Work out the finished part from the listing and answer in its coordinate system (mm). Round coordinates to 2 decimals unless told otherwise and drop trailing zeros. Order: outer loops, then holes, each group sorted by start corner. A loop starts at its lowest first (then second) coordinate and runs counter-clockwise, first axis right, second up. Notation, with made-up numbers: (84, 81.5) -> (88, 81.5) arc R36 cw to (88, 118.5) -> close; hole circle Ø6 at (40.5, 8). An arc over 180 degrees is marked (long way). Use one line per item in the form item = value.
```python
from build123d import *

# Parameters (mm, degrees)
SKETCH11_R          = 2.5
MEMBER_1_DEPTH      = 805
CUT_EXTRUDE_1_DEPTH = 404.058618566
HOLE_WIZARD_M6_1_D  = 5


with BuildPart() as part:
    # Sketch11 → Member 1 (new body)
    with BuildSketch(Plane(origin=(-402.5, 0, 0), x_dir=(0, 0, -1), z_dir=(1, 0, 0))):
        with BuildLine():
            Line((-6, -15), (-3.25, -15))
            Line((-3.25, -15), (-3.25, -12.7))
            Line((-3.25, -12.7), (-5, -12.7))
            Line((-5, -12.7), (-5, -7))
            ThreePointArc((-5, -7), (0, -4.31662479), (5, -7))
            Line((5, -7), (5, -12.7))
            Line((5, -12.7), (3.25, -12.7))
            Line((3.25, -12.7), (3.25, -15))
            Line((3.25, -15), (6, -15))
            ThreePointArc((6, -15), (7.060660172, -14.560660172), (7.5, -13.5))
            Line((7.5, -13.5), (7.5, 13.5))
            ThreePointArc((7.5, 13.5), (7.060660172, 14.560660172), (6, 15))
            Line((6, 15), (3.25, 15))
            Line((3.25, 15), (3.25, 12.7))
            Line((3.25, 12.7), (5, 12.7))
            Line((5, 12.7), (5, 7))
            ThreePointArc((5, 7), (0, 4.31662479), (-5, 7))
            Line((-5, 7), (-5, 12.7))
            Line((-5, 12.7), (-3.25, 12.7))
            Line((-3.25, 12.7), (-3.25, 15))
            Line((-3.25, 15), (-6, 15))
            ThreePointArc((-6, 15), (-7.060660172, 14.560660172), (-7.5, 13.5))
            Line((-7.5, 13.5), (-7.5, -13.5))
            ThreePointArc((-7.5, -13.5), (-7.060660172, -14.560660172), (-6, -15))
        make_face()
        Circle(SKETCH11_R, mode=Mode.SUBTRACT)
    extrude(amount=MEMBER_1_DEPTH)

    # 草图4 → 切除-拉伸1 (cut, through all)
    with BuildSketch(Plane.XY.offset(7.5)):
        Polygon((-402.5, 15), (-372.5, -15), (-402.5, -15), align=None)
        Polygon((402.5, -15), (402.5, 15), (372.5, -15), align=None)
    extrude(amount=-CUT_EXTRUDE_1_DEPTH, mode=Mode.SUBTRACT)

    # M6 螺纹孔1 (through all)
    with Locations(Plane.XY.offset(7.5)):
        with Locations((-45, 0), (45, 0)):
            Hole(HOLE_WIZARD_M6_1_D / 2)


solid = part.part
```
Item 1: The part is cut by section A-A, the plane x = 252.5. Give the vertices of the cut face in (y, z).
Findings:
outline = (-15, -6) arc R1.5 ccw to (-13.5, -7.5) -> (13.5, -7.5) arc R1.5 ccw to (15, -6) -> (15, -3.25) -> (12.7, -3.25) -> (12.7, -5) -> (7, -5) arc R6 cw to (7, 5) -> (12.7, 5) -> (12.7, 3.25) -> (15, 3.25) -> (15, 6) arc R1.5 ccw to (13.5, 7.5) -> (-13.5, 7.5) arc R1.5 ccw to (-15, 6) -> (-15, 3.25) -> (-12.7, 3.25) -> (-12.7, 5) -> (-7, 5) arc R6 cw to (-7, -5) -> (-12.7, -5) -> (-12.7, -3.25) -> (-15, -3.25) -> close; hole circle Ø5 at (0, 0)
Item 2: Consider line 1 along Z through (x, y) = (-5, 9.5); line 2 along X through (y, z) = (0, 5.25); line 3 along Y through (x, z) = (-195, 3.75). Determine where each line is inside the solid, lowest interval first.
Findings:
line_1 = -7.5 to -5, 5 to 7.5
line_2 = -387.5 to -47.5, -42.5 to 42.5, 47.5 to 387.5
line_3 = -15 to -12.7, -5.63 to 5.63, 12.7 to 15
Item 3: Flat-ended cylindrical pins translate along their axes: P1, Ø1, axis at x = 196, z = -2.5, coming from the +Y side; P2, Ø4, axis at y = -9, z = 3.5, coming from the -X side; P3, Ø2, axis at y = -0.5, z = -5, coming from the -X side; P4, Ø6, axis at x = 45, y = 0, coming from the -Z side. Find the tip coordinate at first contact, or state that the pin passes through.
Findings:
P1 = 5.12
P2 = -379.82
P3 = -388
P4 = -7.5
